For this review, take the finished solid that the model builds, in its own axes (mm). Round coordinates to 2 decimals unless told otherwise and drop trailing zeros. Loops run counter-clockwise (first coordinate to the right, second up) from the corner with the lowest first, then second, coordinate; pieces in that order, holes last.
1. Clearance check with flat-ended pins moving along their axes: pin 1 Ø3.5 at (x, z) = (0, 17.25) entering from -Y; pin 2 Ø7 at (x, z) = (15, 17.25) entering from -Y; pin 3 Ø5 at (x, z) = (0, -17.25) entering from -Y. State where each tip first meets the part, or that it passes through.
2. Consider section B-B on z = -17.25. State the section outline as (x, y) points, then the cut area to 3 significant figures.
3. Draft analysis for pull direction X (two halves, no side actions). For faces 1 (the flat face through (25, 1, 0)), 2 (the cylindrical face through (-13.962, 2.532, -15.254)), 3 (the flat face through (0, 1, -22.5)), state which applies: released by +X, released by -X, zero draft, split by the parting line, or undercut.
4. To check wall thickness, follow line 1 along X through (y, z) = (2.55, 17.25); line 2 along Z through (x, y) = (15, 2.75); line 3 along Z through (x, y) = (12.5, 1.3). State the ranges of each line that lie inside material, in increasing order.
5. Consider section C-C on y = 1.1. State the section outline as (x, z) points.
6. Consider section A-A on x = 15. State the section outline as (y, z) points.
from build123d import *

# Parameters (mm, degrees)
SKETCH_1_W                = 50
SKETCH_1_H                = 45
EXTRUDE_1_DEPTH           = 3
HOLE_WIZARD_1_D           = 4.5
HOLE_WIZARD_1_DEPTH       = 12.4
HOLE_WIZARD_1_CSINK_D     = 8.6
HOLE_WIZARD_1_CSINK_ANGLE = 90
HOLE_WIZARD_1_TIP         = 1.351936393
CHAMFER_1_SIZE            = 3


with BuildPart() as part:
    # 草图1 → 凸台-拉伸1 (new body)
    with BuildSketch(Plane(origin=(0, 0, 0), x_dir=(1, 0, 0), z_dir=(0, 1, 0))):
        Rectangle(SKETCH_1_W, SKETCH_1_H)
    extrude(amount=EXTRUDE_1_DEPTH)

    # 打孔尺寸(%根据)开槽半沉头木螺钉的类型1
    with Locations(Plane(origin=(0, 0, 0), x_dir=(-1, 0, 0), z_dir=(0, -1, 0))):
        with Locations((15, 17.25), (0, 17.25), (-15, 17.25), (-15, -17.25), (0, -17.25), (15, -17.25)):
            CounterSinkHole(HOLE_WIZARD_1_D / 2, HOLE_WIZARD_1_CSINK_D / 2, depth=HOLE_WIZARD_1_DEPTH, counter_sink_angle=HOLE_WIZARD_1_CSINK_ANGLE)
            with Locations((0, 0, -(HOLE_WIZARD_1_DEPTH + HOLE_WIZARD_1_TIP / 2))):  # 118° drill point
                Cone(0, HOLE_WIZARD_1_D / 2, HOLE_WIZARD_1_TIP, mode=Mode.SUBTRACT)

    # 倒角1
    chamfer_1_edges = [part.edges().sort_by_distance(p)[0] for p in [
        (25, 1.5, 22.5),
        (-25, 1.5, 22.5),
        (-25, 1.5, -22.5),
        (25, 1.5, -22.5),
    ]]
    chamfer(chamfer_1_edges, length=CHAMFER_1_SIZE)


solid = part.part
Resolved:
1. pin 1: passes through
1. pin 2: stops at y = 0.8
1. pin 3: stops at y = 1.8
2. outline: (-25, 0) - (-19.3, 0) - (-17.25, 2.05) - (-17.25, 3) - (-25, 3) - close; (-12.75, 2.05) - (-10.7, 0) - (-4.3, 0) - (-2.25, 2.05) - (-2.25, 3) - (-12.75, 3) - close; (2.25, 2.05) - (4.3, 0) - (10.7, 0) - (12.75, 2.05) - (12.75, 3) - (2.25, 3) - close; (17.25, 2.05) - (19.3, 0) - (25, 0) - (25, 3) - (17.25, 3) - close
2. area: 96.9 mm2
3. face 1: released by +X
3. face 2: undercut
3. face 3: zero draft
4. line 1: x = -25 to -17.25, -12.75 to -2.25, 2.25 to 12.75, 17.25 to 25
4. line 2: z = -22.5 to -19.5, -15 to 15, 19.5 to 22.5
4. line 3: z = -22.5 to -18.91, -15.59 to 15.59, 18.91 to 22.5
5. outline: (-25, -19.5) - (-22, -22.5) - (22, -22.5) - (25, -19.5) - (25, 19.5) - (22, 22.5) - (-22, 22.5) - (-25, 19.5) - close; hole circle Ø6.4 at (-15, -17.25); hole circle Ø6.4 at (-15, 17.25); hole circle Ø6.4 at (0, -17.25); hole circle Ø6.4 at (0, 17.25); hole circle Ø6.4 at (15, -17.25); hole circle Ø6.4 at (15, 17.25)
6. outline: (0, -22.5) - (3, -22.5) - (3, -19.5) - (2.05, -19.5) - (0, -21.55) - close; (0, -12.95) - (2.05, -15) - (3, -15) - (3, 15) - (2.05, 15) - (0, 12.95) - close; (0, 21.55) - (2.05, 19.5) - (3, 19.5) - (3, 22.5) - (0, 22.5) - close
